```python
from build123d import *

# Parameters (mm, degrees)
SKETCH1_W                                  = 46
SKETCH1_H                                  = 10
BOSS_EXTRUDE1_DEPTH                        = 48
SKETCH2_W                                  = 16
SKETCH2_H                                  = 5
CUT_EXTRUDE1_DEPTH                         = 10
FILLET1_R                                  = 2
CBORE_FOR_M4_CHEESE_HEAD_SCREW1_AT_2_COUNT = 2
CBORE_FOR_M4_CHEESE_HEAD_SCREW1_AT_2_PITCH = 28
CBORE_FOR_M4_CHEESE_HEAD_SCREW1_AT_3_COUNT = 2
CBORE_FOR_M4_CHEESE_HEAD_SCREW1_AT_3_PITCH = 41.036569057
CBORE_FOR_M4_CHEESE_HEAD_SCREW1_AT_4_COUNT = 2
CBORE_FOR_M4_CHEESE_HEAD_SCREW1_AT_4_PITCH = 30
SKETCH6_R                                  = 7
CUT_EXTRUDE2_DEPTH                         = 5


with BuildPart() as part:
    # Sketch1 → Boss-Extrude1 (new body)
    with BuildSketch(Plane.XY):
        Rectangle(SKETCH1_W, SKETCH1_H)
    extrude(amount=BOSS_EXTRUDE1_DEPTH)

    # Sketch2 → Cut-Extrude1 (cut)
    with BuildSketch(Plane(origin=(0, 5, 0), x_dir=(1, 0, 0), z_dir=(0, 1, 0))):
        with Locations((0, -48)):
            Rectangle(SKETCH2_W, SKETCH2_H)
        Rectangle(SKETCH2_W, SKETCH2_H)
    extrude(amount=-CUT_EXTRUDE1_DEPTH, mode=Mode.SUBTRACT)

    # Fillet1
    fillet1_edges = [part.edges().sort_by_distance(p)[0] for p in [
        (-8, 0, 0),
        (8, 0, 0),
        (8, 0, 48),
        (-8, 0, 48),
    ]]
    fillet(fillet1_edges, radius=FILLET1_R)

    # Sketch4 → CBORE for M4 Cheese Head Screw1 (revolve, cut)
    with BuildSketch(Plane(origin=(-15, 5, 10), x_dir=(0, 0, 1), z_dir=(1, 0, 0))):
        Polygon((0, 0), (0, 11.351936393), (2.25, 10), (2.25, 2.6), (4, 2.6), (4, 0.025), (4.025, 0), align=None)
    cbore_for_m4_cheese_head_screw1 = revolve(axis=Axis((-15, 11.35, 10), (0, -1, 0)), mode=Mode.SUBTRACT)

    # CBORE for M4 Cheese Head Screw1 at 2: CBORE for M4 Cheese Head Screw1 ×2
    with Locations(*[(0, 0, i * CBORE_FOR_M4_CHEESE_HEAD_SCREW1_AT_2_PITCH) for i in range(1, CBORE_FOR_M4_CHEESE_HEAD_SCREW1_AT_2_COUNT)]):
        add(cbore_for_m4_cheese_head_screw1, mode=Mode.SUBTRACT)

    # CBORE for M4 Cheese Head Screw1 at 3: CBORE for M4 Cheese Head Screw1 ×2
    with Locations(*[Vector(0.731055268242869, 0, 0.6823182503600111) * (i * CBORE_FOR_M4_CHEESE_HEAD_SCREW1_AT_3_PITCH) for i in range(1, CBORE_FOR_M4_CHEESE_HEAD_SCREW1_AT_3_COUNT)]):
        add(cbore_for_m4_cheese_head_screw1, mode=Mode.SUBTRACT)

    # CBORE for M4 Cheese Head Screw1 at 4: CBORE for M4 Cheese Head Screw1 ×2
    with Locations(*[(i * CBORE_FOR_M4_CHEESE_HEAD_SCREW1_AT_4_PITCH, 0, 0) for i in range(1, CBORE_FOR_M4_CHEESE_HEAD_SCREW1_AT_4_COUNT)]):
        add(cbore_for_m4_cheese_head_screw1, mode=Mode.SUBTRACT)

    # Sketch6 → Cut-Extrude2 (cut)
    with BuildSketch(Plane(origin=(0, 5, 0), x_dir=(1, 0, 0), z_dir=(0, 1, 0))):
        with Locations(Location((0, -24, 0), (0, 0, 270))):
            Circle(SKETCH6_R)
    extrude(amount=-CUT_EXTRUDE2_DEPTH, mode=Mode.SUBTRACT)


solid = part.part
```
The model under review builds one solid part; all positions refer to its coordinate system, in mm. A direction names the side the tool comes from. Round coordinates to 2 decimals unless told otherwise and drop trailing zeros. Order: outer loops, then holes, each group sorted by start corner. A loop starts at its lowest first (then second) coordinate and runs counter-clockwise, first axis right, second up. Notation, with made-up numbers: M 86,74.5 L 91,74.5 A31 cw 91,106.5 Z; hole C -30,-9.5 d11. An arc over 180 degrees is marked long. Use a Markdown table: item, result.
1) Insertion check: pin 1 (3 mm diameter, centred on x = -3.5, y = 3.5, fed in from +Z); pin 2 (5 mm diameter, centred on x = 15, z = 38, fed in from +Y); pin 3 (13 mm diameter, centred on x = 15, z = 10, fed in from +Y); pin 4 (3 mm diameter, centred on x = -1.5, y = 1, fed in from -Z). Each pin has a flat end and moves straight along its axis. Give the tip position at first contact, or say it passes through.
Report:
| item | result |
|---|---|
| pin 1 | z = 45.5 |
| pin 2 | y = 2.4 |
| pin 3 | y = 5 |
| pin 4 | z = 2.5 |
2) Consider section D-D (x = 0). Write out the cut boundary in (y, z), then the cut area to 3 significant figures.
Report:
| item | result |
|---|---|
| outline | M -5,2.5 L 5,2.5 L 5,17 L 0,17 L 0,31 L 5,31 L 5,45.5 L -5,45.5 Z |
| area | 360 mm^2 |
3) Consider section C-C (y = -3.25). Write out the cut boundary in (x, z).
Report:
| item | result |
|---|---|
| outline | M -23,0 L -10,0 A2 ccw -8,2 L -8,2.5 L 8,2.5 L 8,2 A2 ccw 10,0 L 23,0 L 23,48 L 10,48 A2 ccw 8,46 L 8,45.5 L -8,45.5 L -8,46 A2 ccw -10,48 L -23,48 Z; hole C -15,10 d4.5; hole C -15,38 d4.5; hole C 15,10 d4.5; hole C 15,38 d4.5 |
4) Tool access review of faces 1 (the face through (23, 0, 24)), 2 (the face through (-13, 2.4, 36)), 3 (the face through (-8.6, 0.07, 0.57)), 4 (the face through (-12.804, -1.248, 9.512)), 5 (the face through (8.6, 0.07, 47.43)): name each direction out of +Z, -Z, +X, -X, +Y, -Y from which nothing blocks a thin tool from reaching the whole face with its end or side.
Report:
| item | result |
|---|---|
| face 1 | +Z, -Z, +X, +Y, -Y |
| face 2 | +Y |
| face 3 | -Z, +Y, -Y |
| face 4 | +Y, -Y |
| face 5 | +Z, +Y, -Y |
5) Consider section A-A (x = -15). Write out the cut boundary in (y, z) (3 decimals).
Report:
| item | result |
|---|---|
| outline | M -5,0 L 5,0 L 5,5.975 L 4.975,6 L 2.4,6 L 2.4,7.75 L -5,7.75 Z; M -5,12.25 L 2.4,12.25 L 2.4,14 L 4.975,14 L 5,14.025 L 5,33.975 L 4.975,34 L 2.4,34 L 2.4,35.75 L -5,35.75 Z; M -5,40.25 L 2.4,40.25 L 2.4,42 L 4.975,42 L 5,42.025 L 5,48 L -5,48 Z |
6) Wall thickness on line 1 along Z through (x, y) = (15, -0.5); line 2 along X through (y, z) = (-3, 10); line 3 along Z through (x, y) = (15, 4.5): over which ranges is each line inside the solid? List them lowest first. Write a range as [from, to].
Report:
| item | result |
|---|---|
| line 1 | [0, 7.75], [12.25, 35.75], [40.25, 48] |
| line 2 | [-23, -17.25], [-12.75, 12.75], [17.25, 23] |
| line 3 | [0, 6], [14, 34], [42, 48] |
7) Draft analysis for pull direction Z (two halves, no side actions). For faces 6 (the face through (14.901, -1.248, 35.752)), 7 (the face through (-17, 0, 0)), 8 (the face through (-17, 0, 48)), state which applies: released by +Z, released by -Z, zero draft, split by the parting line, or undercut.
Report:
| item | result |
|---|---|
| face 6 | undercut |
| face 7 | released by -Z |
| face 8 | released by +Z |
8) Consider section B-B (z = 38). Write out the cut boundary in (x, y) (3 decimals).
Report:
| item | result |
|---|---|
| outline | M -23,-5 L -17.25,-5 L -17.25,2.4 L -19,2.4 L -19,4.975 L -19.025,5 L -23,5 Z; M -12.75,-5 L 12.75,-5 L 12.75,2.4 L 11,2.4 L 11,4.975 L 10.975,5 L -10.975,5 L -11,4.975 L -11,2.4 L -12.75,2.4 Z; M 17.25,-5 L 23,-5 L 23,5 L 19.025,5 L 19,4.975 L 19,2.4 L 17.25,2.4 Z |
